from build123d import *

# Parameters (mm, degrees)
BASE_PLATE_DEPTH      = 10
SUPPORT_BOSS_SKETCH_R = 6.810683872
SUPPORT_BOSS_DEPTH    = 70
FLANGE_DEPTH          = 12
FLANGE_SLOT_SKETCH_R  = 7.5
FLANGE_SLOT_CUT_DEPTH = 12


with BuildPart() as part:
    # Base Plate Sketch → Base Plate (new body)
    with BuildSketch(Plane(origin=(0, 0, 0), x_dir=(1, 0, 0), z_dir=(0, 1, 0))):
        with BuildLine():
            Line((0, 0), (47, 0))
            ThreePointArc((47, 0), (57.606601718, 4.393398282), (62, 15))
            Line((62, 15), (62, 25))
            Line((62, 25), (47, 25))
            ThreePointArc((47, 25), (37, 35), (47, 45))
            Line((47, 45), (62, 45))
            Line((62, 45), (62, 55))
            ThreePointArc((62, 55), (57.606601718, 65.606601718), (47, 70))
            Line((47, 70), (0, 70))
            Line((0, 70), (0, 0))
        make_face()
    extrude(amount=BASE_PLATE_DEPTH)

    # Support Boss Sketch → Support Boss (add, through all)
    with BuildSketch(Plane.XY):
        with BuildLine():
            Line((0, 0), (0, -30))
            ThreePointArc((0, -30), (10, -40), (20, -30))
            Line((20, -30), (20, -5))
            ThreePointArc((20, -5), (21.464466094, -1.464466094), (25, 0))
            Line((25, 0), (0, 0))
        make_face()
        with Locations((10, -30)):
            Circle(SUPPORT_BOSS_SKETCH_R, mode=Mode.SUBTRACT)
    extrude(amount=-SUPPORT_BOSS_DEPTH)

    # Flange Sketch → Flange (add)
    with BuildSketch(Plane.ZY):
        with BuildLine():
            Line((-70, 10), (-70, 42.5))
            ThreePointArc((-70, 42.5), (-57.5, 55), (-45, 42.5))
            ThreePointArc((-45, 42.5), (-43.535533906, 38.964466094), (-40, 37.5))
            Line((-40, 37.5), (-30, 37.5))
            ThreePointArc((-30, 37.5), (-26.464466094, 38.964466094), (-25, 42.5))
            ThreePointArc((-25, 42.5), (-12.5, 55), (0, 42.5))
            Line((0, 42.5), (0, 10))
            Line((0, 10), (-70, 10))
        make_face()
    extrude(amount=-FLANGE_DEPTH)

    # Flange Slot Sketch → Flange Slot Cut (cut)
    with BuildSketch(Plane(origin=(12, 0, 0), x_dir=(0, 0, -1), z_dir=(1, 0, 0))):
        with Locations((12.5, 42.5)):
            Circle(FLANGE_SLOT_SKETCH_R)
        with Locations((57.5, 42.5)):
            Circle(FLANGE_SLOT_SKETCH_R)
    extrude(amount=-FLANGE_SLOT_CUT_DEPTH, mode=Mode.SUBTRACT)


solid = part.part
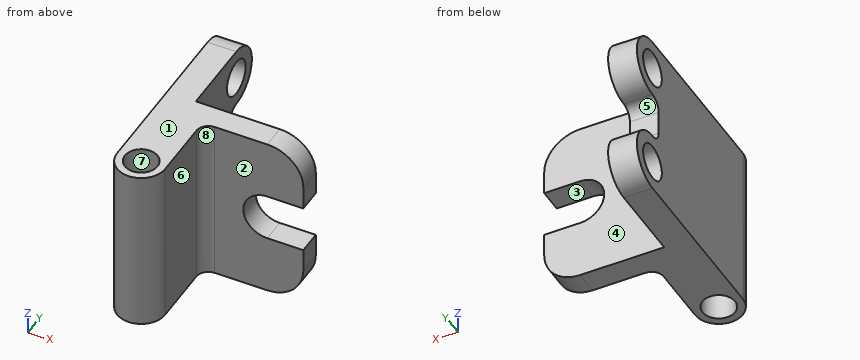
Model file for the job. Use its own axes, mm. Face numbers are marked on the shaded views. A direction names the side the tool comes from. Round coordinates to 2 decimals unless told otherwise and drop trailing zeros. Order: outer loops, then holes, each group sorted by start corner. A loop starts at its lowest first (then second) coordinate and runs counter-clockwise, first axis right, second up.
(1) Drill centre lines: line 1 (Y direction, x = 5, z = -12); line 2 (Y direction, x = 4.25, z = -12.5); line 3 (X direction, y = 24, z = -38). Where is each one in solid material? Low to high.
(2) 3-axis set-ups, long thin cutter, end or side, ignore diameter. For the marked faces 1, 2, 3 and 4: which of +Z, -Z, +X, -X, +Y, -Y reach the whole face in a straight line?
(3) Pin check, flat tips, straight feed: pin 1 (4 mm diameter, centred on y = -3, z = -62, fed in from -X); pin 2 (11 mm diameter, centred on x = 53, y = 5.5, fed in from +Z); pin 3 (5 mm diameter, centred on x = 54, y = 5, fed in from -Z); pin 4 (11 mm diameter, centred on x = 6.5, z = -37, fed in from +Y). Stop position of each tip, or through.
(4) Band-saw the part on B-B (z = -12.5). List the corners of the cut face in (x, y).
(5) Band-saw the part on C-C (y = 45.5). List the corners of the cut face in (x, z).
(6) Band-saw the part on A-A (x = 10). List the corners of the cut face in (y, z).
(7) Pull direction Y, two halves, no side cores. Call the marked faces 5, 6, 7 and 8: released by +Y, released by -Y, zero draft, split by the parting line, or undercut.
(8) Band-saw the part on D-D (x = 51.5). List the corners of the cut face in (y, z), then the cut area to 3 significant figures.
Verdict:
1. line 1: y = -38.66 to -34.62, -25.38 to 35.02, 49.98 to 54.99
1. line 2: y = -38.18 to -33.65, -26.35 to 35, 50 to 55
1. line 3: x = 0 to 12
2. face 1: +Z, +X, -X, +Y, -Y
2. face 2: +Z, -Z, +X, -Y
2. face 3: +X, +Y, -Y
2. face 4: +Z, -Z, +X, +Y
3. pin 1: stops at x = 0
3. pin 2: stops at z = -0.01
3. pin 3: stops at z = -69.31
3. pin 4: stops at y = 38.17
4. outline: (0, -30) arc R10 ccw to (20, -30) - (20, -5) arc R5 cw to (25, 0) - (61.79, 0) - (61.79, 10) - (12, 10) - (12, 35) - (0, 35) - close; (0, 50) - (12, 50) - (12, 55) - (0, 55) - close; hole circle Ø13.62 at (10, -30)
5. outline: (0, -69.63) - (12, -69.63) - (12, -64.37) - (0, -64.37) - close; (0, -50.63) - (12, -50.63) - (12, -45.37) - (0, -45.37) - close; (0, -24.63) - (12, -24.63) - (12, -19.37) - (0, -19.37) - close; (0, -5.63) - (12, -5.63) - (12, -0.37) - (0, -0.37) - close
6. outline: (-40, -70) - (-36.81, -70) - (-36.81, 0) - (-40, 0) - close; (-23.19, -70) - (42.5, -70) arc R12.5 ccw to (42.5, -45) arc R5 cw to (37.5, -40) - (37.5, -30) arc R5 cw to (42.5, -25) arc R12.5 ccw to (42.5, 0) - (-23.19, 0) - close; hole circle Ø15 at (42.5, -57.5); hole circle Ø15 at (42.5, -12.5)
7. face 5: released by +Y
7. face 6: zero draft
7. face 7: undercut
7. face 8: released by -Y
8. outline: (0, -69.31) - (10, -69.31) - (10, -45) - (0, -45) - close; (0, -25) - (10, -25) - (10, -0.69) - (0, -0.69) - close
8. area: 486 mm2
